Study the drawing (mm; zero at the part's minimum x, y, z) and answer. A direction names the side the tool comes from. Round coordinates to 2 decimals unless told otherwise and drop trailing zeros. Loops run counter-clockwise (first coordinate to the right, second up) from the corner with the lowest first, then second, coordinate; pieces in that order, holes last. Notation, with made-up numbers: (44.25, 28) -> (49.25, 28) arc R24 cw to (49.25, 47) -> close; hole circle Ø4 at (26, 16). An arc over 180 degrees is marked (long way). Write each question's results on one line, items separated by ' | '. Start each with the question number.
(1) Straight lines are drawn through the part: probe 1 along X at (y, z) = (7, 34); probe 2 along X at (y, z) = (9.75, 54); probe 3 along Y at (x, z) = (16.5, 57.5). For each, find the intervals that lie inside material, in ascending order.
(2) The part is cut by section C-C (z = 59). Determine the outline of the cut face in (x, y), plus the area to 3 significant figures.
(3) The part is cut by section D-D (y = 4.75). Determine the outline of the cut face in (x, z), plus the area to 3 significant figures.
(4) Flat-ended cylindrical pins translate along their axes: pin 1 (8 mm diameter, centred on x = 13.5, z = 32, fed in from +Y); pin 2 (1 mm diameter, centred on x = 58.5, y = 11.5, fed in from -Z); pin 3 (2 mm diameter, centred on x = 6, y = 11.5, fed in from +Z); pin 4 (6.5 mm diameter, centred on x = 34, z = 9, fed in from -Y). Find the tip coordinate at first contact, or state that the pin passes through.
(5) For the marked faces 1, 2 and 3, determine the directions among +Z, -Z, +X, -X, +Y, -Y from which every point of the face is accessible in a straight line to the end or side of a thin tool.
(6) The part is cut by section B-B (x = 34). Determine the outline of the cut face in (y, z), plus the area to 3 significant figures.
(7) Determine the mould class of the marked faces 4, 5, 6 and 7 for opening direction Z: released by +Z, released by -Z, zero draft, split by the parting line, or undercut.
(8) The part is cut by section A-A (z = 34). Determine the outline of the cut face in (x, y), plus the area to 3 significant figures.
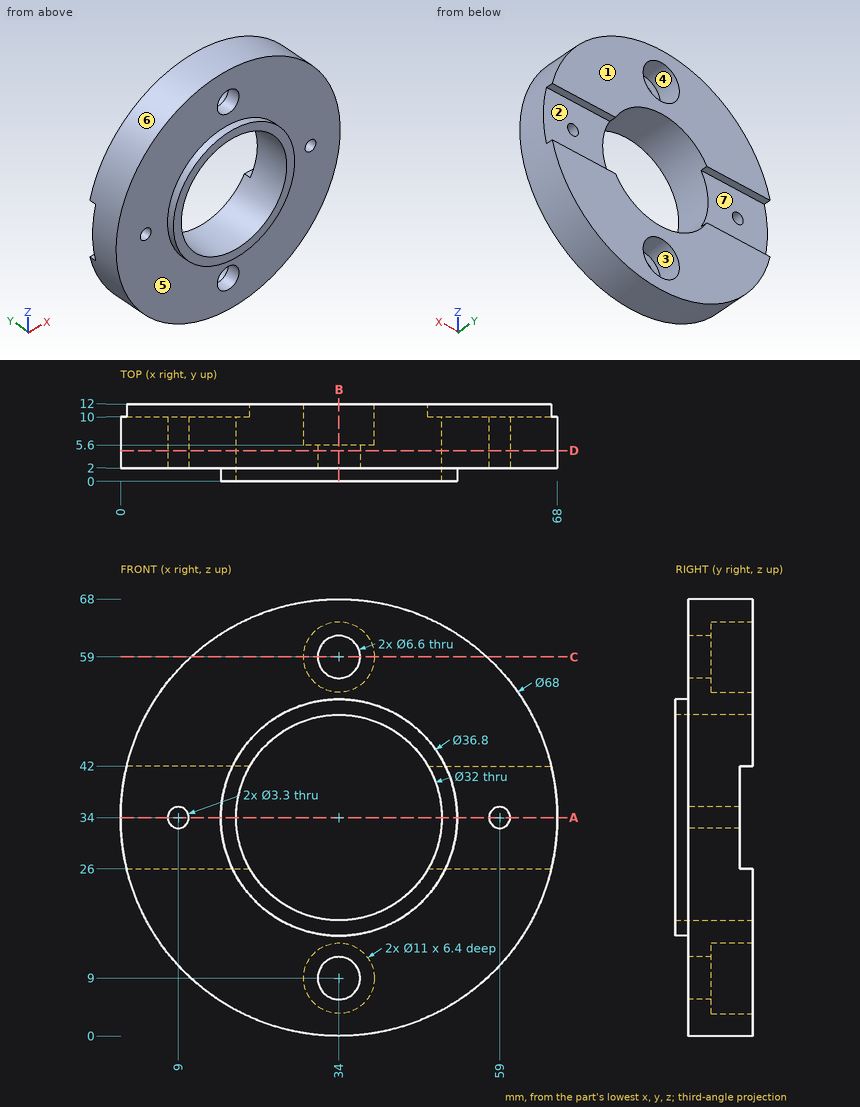
Checked values:
1) probe 1: x = 0 to 7.35, 10.65 to 18, 50 to 57.35, 60.65 to 68 | probe 2: x = 6.5 to 31.71, 36.29 to 61.5 | probe 3: y = 2 to 12
2) outline: (10.96, 2) -> (30.7, 2) -> (30.7, 5.6) -> (28.5, 5.6) -> (28.5, 12) -> (10.96, 12) -> close; (37.3, 2) -> (57.04, 2) -> (57.04, 12) -> (39.5, 12) -> (39.5, 5.6) -> (37.3, 5.6) -> close | area: 367 mm2
3) outline: circle Ø68 at (34, 34); hole circle Ø3.3 at (9, 34); hole circle Ø32 at (34, 34); hole circle Ø6.6 at (34, 9); hole circle Ø6.6 at (34, 59); hole circle Ø3.3 at (59, 34) | area: 2,740 mm2
4) pin 1: stops at y = 10 | pin 2: stops at z = 9.92 | pin 3: stops at z = 54.66 | pin 4: passes through
5) face 1: +Z, -Z, +X, -X, +Y | face 2: +X, -X, +Y | face 3: +Y
6) outline: (0, 15.6) -> (2, 15.6) -> (2, 12.3) -> (5.6, 12.3) -> (5.6, 14.5) -> (12, 14.5) -> (12, 18) -> (0, 18) -> close; (0, 50) -> (12, 50) -> (12, 53.5) -> (5.6, 53.5) -> (5.6, 55.7) -> (2, 55.7) -> (2, 52.4) -> (0, 52.4) -> close; (2, 0) -> (12, 0) -> (12, 3.5) -> (5.6, 3.5) -> (5.6, 5.7) -> (2, 5.7) -> close; (2, 62.3) -> (5.6, 62.3) -> (5.6, 64.5) -> (12, 64.5) -> (12, 68) -> (2, 68) -> close | area: 181 mm2
7) face 4: undercut | face 5: zero draft | face 6: split by the parting line | face 7: undercut
8) outline: (0, 2) -> (7.35, 2) -> (7.35, 10) -> (0, 10) -> close; (10.65, 2) -> (15.6, 2) -> (15.6, 0) -> (18, 0) -> (18, 10) -> (10.65, 10) -> close; (50, 0) -> (52.4, 0) -> (52.4, 2) -> (57.35, 2) -> (57.35, 10) -> (50, 10) -> close; (60.65, 2) -> (68, 2) -> (68, 10) -> (60.65, 10) -> close | area: 245 mm2
